Geometry: final body of the model. Coordinates: model frame, mm. A direction names the side the tool comes from. Coordinates: 2 decimals unless noted, no trailing zeros. Write each loop counter-clockwise with the first axis right and the second up, starting at its lowest first coordinate (ties: lowest second). Pieces come first, ordered by that corner, then holes. Notation, with made-up numbers: (-10, 5) - (33, 5) arc R28 cw to (33, 35) - close; hole circle Ø10 at (70, 44.5). An arc over 180 degrees is marked (long way). Put each result on its own line as item: value.
```python
from build123d import *

# Parameters (mm, degrees)
BASE_PLATE_DEPTH            = 7.5
PORT_BOSS_SKETCH_R          = 15
QUAD_PORT_BOSS_DEPTH        = 17.5
BOSS_FILLET_R3_A_R          = 3
BOSS_FILLET_R3_B_R          = 3
BOSS_FILLET_R3_C_R          = 3
BOSS_FILLET_R3_D_R          = 3
BOSS_FILLET_R3_E_R          = 3
BOSS_FILLET_R3_F_R          = 3
BOSS_FILLET_R3_G_R          = 3
CENTRAL_CAVITY_SKETCH_R     = 10
CENTRAL_CAVITY_DEPTH        = 17.5
PLATE_CORNER_FILLET_R15_A_R = 15
PLATE_CORNER_FILLET_R15_B_R = 15
PLATE_CORNER_FILLET_R15_C_R = 15
PLATE_CORNER_FILLET_R15_D_R = 15
MOUNTING_HOLES_SKETCH_R     = 5
MOUNTING_HOLES_4X_DEPTH     = 17.5


with BuildPart() as part:
    # Base Plate Sketch → Base Plate (new body)
    with BuildSketch(Plane(origin=(0, 0, 0), x_dir=(1, 0, 0), z_dir=(0, 1, 0))):
        Polygon((40, 0), (40, 56.5), (-40, 56.5), (-40, -56.5), (40, -56.5), align=None)
    extrude(amount=BASE_PLATE_DEPTH)

    # Port Boss Sketch → Quad Port Boss (add)
    with BuildSketch(Plane(origin=(0, 7.5, 0), x_dir=(1, 0, 0), z_dir=(0, 1, 0))):
        with BuildLine():
            ThreePointArc((8.808525392, 26.35875293), (11.311943753, 19.286200894), (16.245240248, 13.633707509))
            ThreePointArc((16.245240248, 13.633707509), (20.808119068, 14.904279215), (25.539691318, 14.68878064))
            ThreePointArc((25.539691318, 14.68878064), (15.628803473, 21.809040991), (14.289691318, 33.93878064))
            ThreePointArc((14.289691318, 33.93878064), (12.155085718, 29.710580725), (8.808525392, 26.35875293))
        make_face()
        with Locations((22.5, 0)):
            Circle(PORT_BOSS_SKETCH_R)
        with BuildLine():
            ThreePointArc((8.808525392, -26.35875293), (12.155085718, -29.710580725), (14.289691318, -33.93878064))
            ThreePointArc((14.289691318, -33.93878064), (15.628803473, -21.809040991), (25.539691318, -14.68878064))
            ThreePointArc((25.539691318, -14.68878064), (20.808119068, -14.904279215), (16.245240248, -13.633707509))
            ThreePointArc((16.245240248, -13.633707509), (11.311943753, -19.286200894), (8.808525392, -26.35875293))
        make_face()
        with Locations((0, -38.5)):
            Circle(PORT_BOSS_SKETCH_R)
        with BuildLine():
            ThreePointArc((-25.539691318, -14.68878064), (-15.628803473, -21.809040991), (-14.289691318, -33.93878064))
            ThreePointArc((-14.289691318, -33.93878064), (-12.155085718, -29.710580725), (-8.808525392, -26.35875293))
            ThreePointArc((-8.808525392, -26.35875293), (-11.311943753, -19.286200894), (-16.245240248, -13.633707509))
            ThreePointArc((-16.245240248, -13.633707509), (-20.808119068, -14.904279215), (-25.539691318, -14.68878064))
        make_face()
        with Locations((-22.5, 0)):
            Circle(PORT_BOSS_SKETCH_R)
        with BuildLine():
            ThreePointArc((-14.289691318, 33.93878064), (-15.628803473, 21.809040991), (-25.539691318, 14.68878064))
            ThreePointArc((-25.539691318, 14.68878064), (-20.808119068, 14.904279215), (-16.245240248, 13.633707509))
            ThreePointArc((-16.245240248, 13.633707509), (-11.311943753, 19.286200894), (-8.808525392, 26.35875293))
            ThreePointArc((-8.808525392, 26.35875293), (-12.155085718, 29.710580725), (-14.289691318, 33.93878064))
        make_face()
        with Locations((0, 38.5)):
            Circle(PORT_BOSS_SKETCH_R)
    extrude(amount=QUAD_PORT_BOSS_DEPTH)

    # Boss Fillet R3 A
    boss_fillet_r3_a_edges = [part.edges().sort_by_distance(p)[0] for p in [
        (-8.808525392, 16.25, -26.35875293),
    ]]
    fillet(boss_fillet_r3_a_edges, radius=BOSS_FILLET_R3_A_R)

    # Boss Fillet R3 B
    boss_fillet_r3_b_edges = [part.edges().sort_by_distance(p)[0] for p in [
        (8.808525392, 16.25, -26.35875293),
    ]]
    fillet(boss_fillet_r3_b_edges, radius=BOSS_FILLET_R3_B_R)

    # Boss Fillet R3 C
    boss_fillet_r3_c_edges = [part.edges().sort_by_distance(p)[0] for p in [
        (16.245240248, 16.25, -13.633707509),
    ]]
    fillet(boss_fillet_r3_c_edges, radius=BOSS_FILLET_R3_C_R)

    # Boss Fillet R3 D
    boss_fillet_r3_d_edges = [part.edges().sort_by_distance(p)[0] for p in [
        (16.245240248, 16.25, 13.633707509),
    ]]
    fillet(boss_fillet_r3_d_edges, radius=BOSS_FILLET_R3_D_R)

    # Boss Fillet R3 E
    boss_fillet_r3_e_edges = [part.edges().sort_by_distance(p)[0] for p in [
        (-16.245240248, 16.25, -13.633707509),
    ]]
    fillet(boss_fillet_r3_e_edges, radius=BOSS_FILLET_R3_E_R)

    # Boss Fillet R3 F
    boss_fillet_r3_f_edges = [part.edges().sort_by_distance(p)[0] for p in [
        (-8.808525392, 16.25, 26.35875293),
    ]]
    fillet(boss_fillet_r3_f_edges, radius=BOSS_FILLET_R3_F_R)

    # Boss Fillet R3 G
    boss_fillet_r3_g_edges = [part.edges().sort_by_distance(p)[0] for p in [
        (8.808525392, 16.25, 26.35875293),
    ]]
    fillet(boss_fillet_r3_g_edges, radius=BOSS_FILLET_R3_G_R)

    # Central Cavity Sketch → Central Cavity (cut)
    with BuildSketch(Plane(origin=(0, 25, 0), x_dir=(1, 0, 0), z_dir=(0, 1, 0))):
        with Locations(Location((0, 38.5, 0), (0, 0, 270))):
            Circle(CENTRAL_CAVITY_SKETCH_R)
        with Locations(Location((22.5, 0, 0), (0, 0, 270))):
            Circle(CENTRAL_CAVITY_SKETCH_R)
        with Locations(Location((0, -38.5, 0), (0, 0, 270))):
            Circle(CENTRAL_CAVITY_SKETCH_R)
        with Locations(Location((-22.5, 0, 0), (0, 0, 270))):
            Circle(CENTRAL_CAVITY_SKETCH_R)
    extrude(amount=-CENTRAL_CAVITY_DEPTH, mode=Mode.SUBTRACT)

    # Plate Corner Fillet R15 A
    plate_corner_fillet_r15_a_edges = [part.edges().sort_by_distance(p)[0] for p in [
        (-40, 3.75, -56.5),
    ]]
    fillet(plate_corner_fillet_r15_a_edges, radius=PLATE_CORNER_FILLET_R15_A_R)

    # Plate Corner Fillet R15 B
    plate_corner_fillet_r15_b_edges = [part.edges().sort_by_distance(p)[0] for p in [
        (40, 3.75, -56.5),
    ]]
    fillet(plate_corner_fillet_r15_b_edges, radius=PLATE_CORNER_FILLET_R15_B_R)

    # Plate Corner Fillet R15 C
    plate_corner_fillet_r15_c_edges = [part.edges().sort_by_distance(p)[0] for p in [
        (40, 3.75, 56.5),
    ]]
    fillet(plate_corner_fillet_r15_c_edges, radius=PLATE_CORNER_FILLET_R15_C_R)

    # Plate Corner Fillet R15 D
    plate_corner_fillet_r15_d_edges = [part.edges().sort_by_distance(p)[0] for p in [
        (-40, 3.75, 56.5),
    ]]
    fillet(plate_corner_fillet_r15_d_edges, radius=PLATE_CORNER_FILLET_R15_D_R)

    # Mounting Holes Sketch → Mounting Holes 4x (cut)
    with BuildSketch(Plane(origin=(0, 7.5, 0), x_dir=(1, 0, 0), z_dir=(0, 1, 0))):
        with Locations(Location((-25, 41.5, 0), (0, 0, 270))):
            Circle(MOUNTING_HOLES_SKETCH_R)
        with Locations(Location((25, 41.5, 0), (0, 0, 270))):
            Circle(MOUNTING_HOLES_SKETCH_R)
        with Locations(Location((25, -41.5, 0), (0, 0, 270))):
            Circle(MOUNTING_HOLES_SKETCH_R)
        with Locations(Location((-25, -41.5, 0), (0, 0, 270))):
            Circle(MOUNTING_HOLES_SKETCH_R)
    extrude(amount=-MOUNTING_HOLES_4X_DEPTH, mode=Mode.SUBTRACT)


solid = part.part
```
1. Section query A-A (z = 38.5). Return loops of the section in (x, y).
Answer below:
outline: (-40, 0) - (-29, 0) - (-29, 7.5) - (-40, 7.5) - close; (-21, 0) - (21, 0) - (21, 7.5) - (15, 7.5) - (15, 25) - (10, 25) - (10, 7.5) - (-10, 7.5) - (-10, 25) - (-15, 25) - (-15, 7.5) - (-21, 7.5) - close; (29, 0) - (40, 0) - (40, 7.5) - (29, 7.5) - close
2. Pin query (flat end, axial travel): pin 1 Ø10 at (x, z) = (23, -4) entering from +Y; pin 2 Ø1.5 at (y, z) = (8.5, -2) entering from +X; pin 3 Ø6 at (x, z) = (-25, -41.5) entering from +Y (3 decimals); pin 4 Ø3 at (y, z) = (18, -26) entering from +X. Return the tip coordinate at first contact, or that it passes through.
Answer below:
pin 1: stops at y = 7.5
pin 2: stops at x = 37.45
pin 3: passes through
pin 4: stops at x = 14.39
3. Set-up query: faces 4 (the flat face through (-1, 7.5, 0)), 5 (the flat face through (40, 4, 1)). Return all of +Z, -Z, +X, -X, +Y, -Y with unobstructed straight access to the full face (end or side cutting, diameter ignored); none if empty.
Answer below:
face 4: +Y
face 5: +Z, -Z, +X, +Y, -Y
4. Mould query, pull axis Z, two halves, no side actions, for faces 1 (the cylindrical face through (-35.49, 3.8, 52.22)), 2 (the cylindrical face through (-0.1, 16.1, -23.5)), 3 (the flat face through (-9, 25, 0)). Classes: +Z half, -Z half, draft (parallel to the pull), parting line (faces both ways), or undercut.
Answer below:
face 1: +Z half
face 2: undercut
face 3: draft
5. Section query C-C (z = -32). Return loops of the section in (x, y), then the cut area to 3 significant figures.
Answer below:
outline: (-40, 0) - (40, 0) - (40, 7.5) - (13.81, 7.5) - (13.81, 25) - (7.6, 25) - (7.6, 7.5) - (-7.6, 7.5) - (-7.6, 25) - (-13.81, 25) - (-13.81, 7.5) - (-40, 7.5) - close
area: 817 mm²
6. Section query D-D (z = -44.5). Return loops of the section in (x, y), then the cut area to 3 significant figures.
Answer below:
outline: (-39.7, 0) - (-29, 0) - (-29, 7.5) - (-39.7, 7.5) - close; (-21, 0) - (21, 0) - (21, 7.5) - (13.75, 7.5) - (13.75, 25) - (8, 25) - (8, 7.5) - (-8, 7.5) - (-8, 25) - (-13.75, 25) - (-13.75, 7.5) - (-21, 7.5) - close; (29, 0) - (39.7, 0) - (39.7, 7.5) - (29, 7.5) - close
area: 677 mm²
7. Section query B-B (y = 5.5). Return loops of the section in (x, z).
Answer below:
outline: (-40, -41.5) arc R15 ccw to (-25, -56.5) - (25, -56.5) arc R15 ccw to (40, -41.5) - (40, 41.5) arc R15 ccw to (25, 56.5) - (-25, 56.5) arc R15 ccw to (-40, 41.5) - close; hole circle Ø10 at (-25, -41.5); hole circle Ø10 at (-25, 41.5); hole circle Ø10 at (25, -41.5); hole circle Ø10 at (25, 41.5)
8. Ray query, probe 1 along X at (y, z) = (2.5, -41.5); probe 2 along Z at (x, y) = (6.5, 9.5); probe 3 along Z at (x, y) = (-28, 3.75). Return the intervals inside material, ascending. Write a range as from..to.
Answer below:
probe 1: x = -40..-30, -20..20, 30..40
probe 2: z = -52.02..-46.1, -30.9..-24.83, 24.83..30.9, 46.1..52.02
probe 3: z = -56.2..-45.5, -37.5..37.5, 45.5..56.2
